```python
from build123d import *

# Parameters (mm, degrees)
CUT_EXTRUDE1_DEPTH = 2.5


with BuildPart() as part:
    # Logo3_bib1 → Revolve1 (revolve)
    with BuildSketch(Plane(origin=(0, 0, 0), x_dir=(-1, 0, 0), z_dir=(0, -1, 0))):
        with BuildLine():
            Line((0, -22), (0, 6))
            Line((0, 6), (4.5, 6))
            ThreePointArc((4.5, 6), (4.853553391, 5.853553391), (5, 5.5))
            Line((5, 5.5), (5, 0))
            Line((5, 0), (3, 0))
            Line((3, 0), (3, -0.01))
            Line((3, -0.01), (2.613425636, -0.01))
            ThreePointArc((2.613425636, -0.01), (2.593729481, -0.026527036), (2.606585234, -0.048793852))
            Line((2.606585234, -0.048793852), (3, -0.191985117))
            Line((3, -0.191985117), (3, -21.5))
            Line((3, -21.5), (2.5, -22))
            Line((2.5, -22), (0, -22))
        make_face()
    revolve(axis=Axis((0, 0, -10.585154653), (0, 0, 1)))

    # Logo3_bib2 → Cut-Extrude1 (cut)
    with BuildSketch(Plane(origin=(0, 0, -6), x_dir=(1, 0, 0), z_dir=(0, 0, -1))):
        Polygon((2.886751346, 0), (1.443375673, 2.5), (-1.443375673, 2.5), (-2.886751346, 0), (-1.443375673, -2.5), (1.443375673, -2.5), align=None)
    extrude(amount=-CUT_EXTRUDE1_DEPTH, mode=Mode.SUBTRACT)


solid = part.part
```
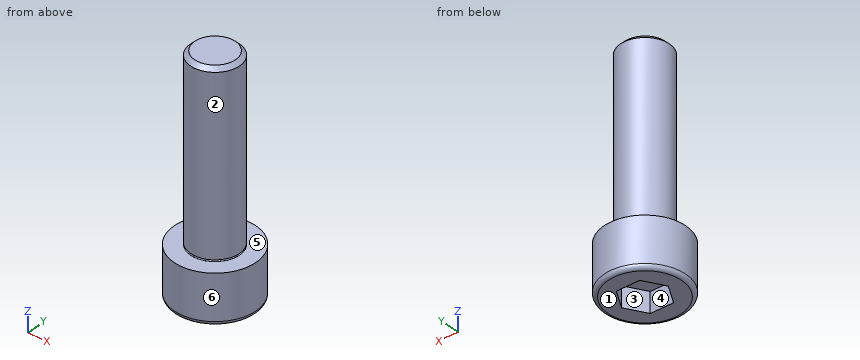
Part model, mm, in its own coordinate system. Face numbers are marked on the shaded views. A direction names the side the tool comes from. Round coordinates to 2 decimals unless told otherwise and drop trailing zeros. Write each loop counter-clockwise with the first axis right and the second up, starting at its lowest first coordinate (ties: lowest second). Pieces come first, ordered by that corner, then holes. Notation, with made-up numbers: M 52.25,-11.5 L 110.25,-11.5 A18 ccw 110.25,13.5 Z; hole C 6.25,-25.75 d6. An arc over 180 degrees is marked long. One line per question, with ' | ' between items.
(1) 3-axis set-ups, long thin cutter, end or side, ignore diameter. For the marked faces 4, 5 and 6: which of +Z, -Z, +X, -X, +Y, -Y reach the whole face in a straight line?
Answer key:
face 4: -Z | face 5: +Z | face 6: +Z, -Z
(2) Saw through at A-A on z = -4. Write the cut outline in (x, y).
Answer key:
outline: C 0,0 d10; hole M -2.89,0 L -1.44,-2.5 L 1.44,-2.5 L 2.89,0 L 1.44,2.5 L -1.44,2.5 Z
(3) Two-plate mould, pull along X, no slides. Class the marked faces 1, 2 and 3: released by +X, released by -X, zero draft, split by the parting line, or undercut.
Answer key:
face 1: zero draft | face 2: split by the parting line | face 3: undercut
(4) Pin check, flat tips, straight feed: pin 1 (4 mm diameter, centred on x = -2.5, z = 11.5, fed in from +Y); pin 2 (1.5 mm diameter, centred on y = -2.5, z = 16, fed in from +X); pin 3 (3 mm diameter, centred on y = -1.5, z = 5, fed in from -X). Stop position of each tip, or through.
Answer key:
pin 1: stops at y = 2.96 | pin 2: stops at x = 2.44 | pin 3: stops at x = -3
(5) Saw through at B-B on z = 6. Write the cut outline in (x, y).
Answer key:
outline: C 0,0 d6
(6) Probe line 1 along Z through (x, y) = (-1, 1); line 2 along Y through (x, z) = (-4, -2.5); line 3 along Z through (x, y) = (-3, -3.25). List the from-to ranges inside material, lowest first.
Answer key:
line 1: z = -3.5 to 22 | line 2: y = -3 to 3 | line 3: z = -6 to 0
